Part model, mm, in its own coordinate system. Face numbers are marked on the shaded views. A direction names the side the tool comes from. Coordinates: 2 decimals unless noted, no trailing zeros. Order: outer loops, then holes, each group sorted by start corner. A loop starts at its lowest first (then second) coordinate and runs counter-clockwise, first axis right, second up. Notation, with made-up numbers: (49, 89.25) - (78, 89.25) arc R18 ccw to (78, 108.25) - close; hole circle Ø3 at (82, 20). An arc over 180 degrees is marked (long way). Use a Markdown table: item, result. Add a question column.
1) Saw through at D-D on x = 0. List the corners of the cut face in (y, z).
2) Saw through at B-B on y = 0. List the corners of the cut face in (x, z), then the cut area to 3 significant figures.
3) Saw through at A-A on z = -21. List the corners of the cut face in (x, y).
4) Two-plate mould, pull along X, no slides. Class the marked faces 6, 7, 8 and 9: +X half, -X half, draft (parallel to the pull), parting line (faces both ways), or undercut.
5) Saw through at C-C on z = -43. List the corners of the cut face in (x, y).
6) Wall check: L1, parallel to X at y = 49, z = -33; L2, parallel to X at y = -4, z = -42; L3, parallel to Y at x = 16, z = -21. Give the ranges that are in metal, low to high. Write a range as [from, to].
7) Tool access for the marked faces 1, 2, 3, 4 and 5: list every direction of +Z, -Z, +X, -X, +Y, -Y with a clear straight run to the whole face (end or side of a thin tool).
8) Drop flat-ended pins along their axis: P1, Ø15, axis at y = 53, z = -25, coming from the -X side; P2, Ø8, axis at y = 38.5, z = -19, coming from the +X side; P3, Ø23, axis at x = -50, y = 0, coming from the -Z side; P4, Ø13.5, axis at y = 54.47, z = -21, coming from the +X side. Give the stop position or say it passes through.
```python
from build123d import *
from build123d.topology import SkipClean

# Parameters (mm, degrees)
HUB_SKETCH_R                   = 35
BEARING_HUB_DEPTH              = 50
BORE_SKETCH_R                  = 20
BEARING_BORE_40_DEPTH          = 71.356236397
MOUNTING_FLANGE_DEPTH          = 12
FLANGE_FILLETS_R8_R            = 8
FLANGE_HOLES_SKETCH_R          = 10
FLANGE_MOUNTING_HOLES_20_DEPTH = 12
CLEVIS_LUG_1_DEPTH             = 10
LUG_1_BOSS_SKETCH_R            = 15
LUG_1_BOSS_30_DEPTH            = 4
CLEVIS_START                   = -10
CLEVIS_LUG_2_DEPTH             = 10
LUG_START                      = 4
LUG_2_BOSS_SKETCH_R            = 15
LUG_2_BOSS_30_DEPTH            = 4
PIN_HOLE_SKETCH_R              = 7.5
LUG_PIN_HOLE_15_DEPTH          = 130.275867818


with BuildPart() as part:
    # Hub Sketch → Bearing Hub (new body)
    with BuildSketch(Plane.XY):
        Circle(HUB_SKETCH_R)
    extrude(amount=-BEARING_HUB_DEPTH)

    # Bore Sketch → Bearing Bore Ø40 (cut, through all)
    with BuildSketch(Plane.XY):
        Circle(BORE_SKETCH_R)
    extrude(amount=-BEARING_BORE_40_DEPTH, mode=Mode.SUBTRACT)

    # Flange Profile Sketch → Mounting Flange (add)
    with BuildSketch(Plane.XY.offset(-38)):
        with BuildLine():
            Line((-50, 20), (-28.722813233, 20))
            ThreePointArc((-28.722813233, 20), (0, -35), (28.722813233, 20))
            Line((28.722813233, 20), (50, 20))
            ThreePointArc((50, 20), (68.47759065, 7.653668647), (64.142135624, -14.142135624))
            Line((64.142135624, -14.142135624), (14.142135624, -64.142135624))
            ThreePointArc((14.142135624, -64.142135624), (0, -70), (-14.142135624, -64.142135624))
            Line((-14.142135624, -64.142135624), (-64.142135624, -14.142135624))
            ThreePointArc((-64.142135624, -14.142135624), (-68.47759065, 7.653668647), (-50, 20))
        make_face()
    extrude(amount=-MOUNTING_FLANGE_DEPTH)

    # Flange Fillets R8
    flange_fillets_r8_edges = [part.edges().sort_by_distance(p)[0] for p in [
        (-28.722813233, 20, -44),
        (28.722813233, 20, -44),
    ]]
    fillet(flange_fillets_r8_edges, radius=FLANGE_FILLETS_R8_R)

    # Flange Holes Sketch → Flange Mounting Holes Ø20 (cut)
    with BuildSketch(Plane.XY.offset(-38)):
        with Locations((50, 0)):
            Circle(FLANGE_HOLES_SKETCH_R)
        with Locations((0, -50)):
            Circle(FLANGE_HOLES_SKETCH_R)
        with Locations((-50, 0)):
            Circle(FLANGE_HOLES_SKETCH_R)
    extrude(amount=-FLANGE_MOUNTING_HOLES_20_DEPTH, mode=Mode.SUBTRACT)

    # Lug 1 Profile Sketch → Clevis Lug 1 (add)
    with BuildSketch(Plane(origin=(12.5, 0, 0), x_dir=(0, 0, -1), z_dir=(1, 0, 0))):
        with BuildLine():
            Line((6, 54.471410374), (6, 26.471410374))
            Line((6, 26.471410374), (36, 26.471410374))
            Line((36, 26.471410374), (36, 54.471410374))
            ThreePointArc((36, 54.471410374), (21, 69.471410374), (6, 54.471410374))
        make_face()
    extrude(amount=CLEVIS_LUG_1_DEPTH)

    # Lug 1 Boss Sketch → Lug 1 Boss Ø30 (add)
    with BuildSketch(Plane(origin=(22.5, 0, 0), x_dir=(0, 0, -1), z_dir=(1, 0, 0))):
        with Locations((21, 54.471410374)):
            Circle(LUG_1_BOSS_SKETCH_R)
    extrude(amount=LUG_1_BOSS_30_DEPTH)

    # Lug 2 Profile Sketch → Clevis Lug 2 (add)
    with BuildSketch(Plane(origin=(-12.5, 0, 0), x_dir=(0, 0, -1), z_dir=(1, 0, 0)).offset(CLEVIS_START)):
        with BuildLine():
            Line((36, 54.471410374), (36, 26.471410374))
            Line((36, 26.471410374), (6, 26.471410374))
            Line((6, 26.471410374), (6, 54.471410374))
            ThreePointArc((6, 54.471410374), (21, 69.471410374), (36, 54.471410374))
        make_face()
    extrude(amount=CLEVIS_LUG_2_DEPTH)

    # Lug 2 Boss Sketch → Lug 2 Boss Ø30 (add)
    with SkipClean():  # the faces are left unmerged after this step: merging them gives an invalid solid
        with BuildSketch(Plane.ZY.offset(22.5).offset(LUG_START)):
            with Locations(Location((-21, 54.471410374, 0), (0, 0, 180))):
                Circle(LUG_2_BOSS_SKETCH_R)
        extrude(amount=-LUG_2_BOSS_30_DEPTH)

    # Pin Hole Sketch → Lug Pin Hole Ø15 (cut, through all)
    with SkipClean():  # the faces are left unmerged after this step: merging them gives an invalid solid
        with BuildSketch(Plane(origin=(26.5, 0, 0), x_dir=(0, 0, -1), z_dir=(1, 0, 0))):
            with Locations((21, 54.471410374)):
                Circle(PIN_HOLE_SKETCH_R)
        extrude(amount=-LUG_PIN_HOLE_15_DEPTH, mode=Mode.SUBTRACT)


solid = part.part
```
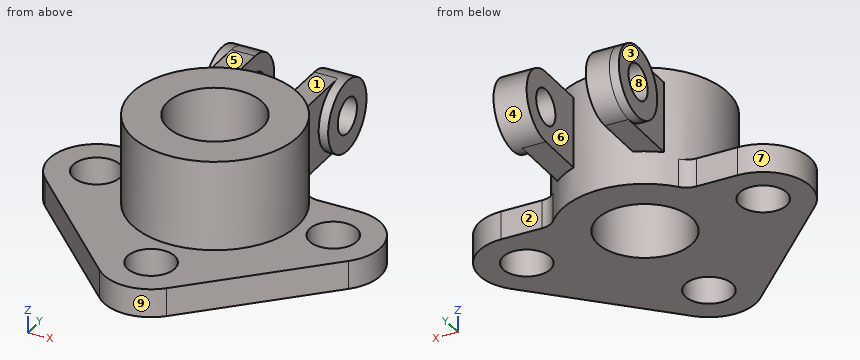
Results are:
| question | item | result |
|---|---|---|
| 1 | outline | (-70, -50) - (-60, -50) - (-60, -38) - (-70, -38) - close; (-40, -50) - (-20, -50) - (-20, 0) - (-35, 0) - (-35, -38) - (-40, -38) - close; (20, -50) - (35, -50) - (35, 0) - (20, 0) - close |
| 2 | outline | (-70, -50) - (-60, -50) - (-60, -38) - (-70, -38) - close; (-40, -50) - (-20, -50) - (-20, 0) - (-35, 0) - (-35, -38) - (-40, -38) - close; (20, -50) - (40, -50) - (40, -38) - (35, -38) - (35, 0) - (20, 0) - close; (60, -50) - (70, -50) - (70, -38) - (60, -38) - close |
| 2 | area | 1,860 mm2 |
| 3 | outline | (-26.5, 39.47) - (-22.5, 39.47) - (-22.5, 26.81) arc R35 ccw (long way) to (22.5, 26.81) - (22.5, 39.47) - (26.5, 39.47) - (26.5, 46.97) - (12.5, 46.97) - (12.5, 32.69) arc R35 ccw to (-12.5, 32.69) - (-12.5, 46.97) - (-26.5, 46.97) - close; (-26.5, 61.97) - (-12.5, 61.97) - (-12.5, 69.47) - (-26.5, 69.47) - close; (12.5, 61.97) - (26.5, 61.97) - (26.5, 69.47) - (12.5, 69.47) - close; hole circle Ø40 at (0, 0) |
| 4 | face 6 | undercut |
| 4 | face 7 | -X half |
| 4 | face 8 | draft |
| 4 | face 9 | parting line |
| 5 | outline | (-64.14, -14.14) - (-14.14, -64.14) arc R20 ccw to (14.14, -64.14) - (64.14, -14.14) arc R20 ccw to (50, 20) - (32.63, 20) arc R8 cw to (26.56, 22.79) arc R35 ccw to (-26.56, 22.79) arc R8 cw to (-32.63, 20) - (-50, 20) arc R20 ccw to start; hole circle Ø20 at (-50, 0); hole circle Ø40 at (0, 0); hole circle Ø20 at (0, -50); hole circle Ø20 at (50, 0) |
| 6 | L1 | [-26.5, -12.5], [12.5, 26.5] |
| 6 | L2 | [-69.6, -59.17], [-40.83, -19.6], [19.6, 40.83], [59.17, 69.6] |
| 6 | L3 | [-31.13, -12], [12, 46.97], [61.97, 69.47] |
| 7 | face 1 | +Z, +X, +Y |
| 7 | face 2 | +Z, -Z, +X, +Y |
| 7 | face 3 | +Z, -Z, -X, +Y |
| 7 | face 4 | +X |
| 7 | face 5 | +Z, -X, +Y |
| 8 | P1 | x = -26.5 |
| 8 | P2 | x = 26.5 |
| 8 | P3 | z = -50 |
| 8 | P4 | through |
